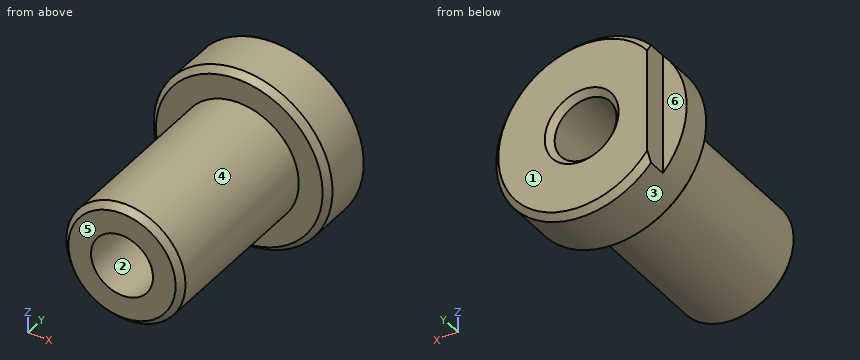
```python
from build123d import *

# Parameters (mm, degrees)
SKETCH1_R           = 5
SKETCH1_R_2         = 2.6
BOSS_EXTRUDE1_DEPTH = 15
SKETCH2_R           = 7.5
SKETCH2_R_2         = 2.6
BOSS_EXTRUDE2_DEPTH = 5
CHAMFER1_SIZE       = 0.5
SKETCH3_W           = 5
SKETCH3_H           = 5
CUT_EXTRUDE1_DEPTH  = 25


with BuildPart() as part:
    # Sketch1 → Boss-Extrude1 (new body)
    with BuildSketch(Plane(origin=(0, 0, 0), x_dir=(1, 0, 0), z_dir=(0, 1, 0))):
        with Locations(Location((0, 0, 0), (0, 0, 270))):
            Circle(SKETCH1_R)
        with Locations(Location((0, 0, 0), (0, 0, 270))):
            Circle(SKETCH1_R_2, mode=Mode.SUBTRACT)
    extrude(amount=BOSS_EXTRUDE1_DEPTH)

    # Sketch2 → Boss-Extrude2 (add)
    with BuildSketch(Plane(origin=(0, 15, 0), x_dir=(1, 0, 0), z_dir=(0, 1, 0))):
        with Locations(Location((0, 0, 0), (0, 0, 270))):
            Circle(SKETCH2_R)
        with Locations(Location((0, 0, 0), (0, 0, 270))):
            Circle(SKETCH2_R_2, mode=Mode.SUBTRACT)
    extrude(amount=BOSS_EXTRUDE2_DEPTH)

    # Chamfer1
    chamfer1_edges = [part.edges().sort_by_distance(p)[0] for p in [
        (0, 20, -7.5),
        (0, 15, -7.5),
        (0, 20, -2.6),
        (0, 0, -5),
    ]]
    chamfer(chamfer1_edges, length=CHAMFER1_SIZE)

    # Sketch3 → Cut-Extrude1 (cut, symmetric)
    with BuildSketch(Plane.XY):
        with Locations((-8, 20.5)):
            Rectangle(SKETCH3_W, SKETCH3_H)
    extrude(amount=CUT_EXTRUDE1_DEPTH, both=True, mode=Mode.SUBTRACT)


solid = part.part
```
CAD build for the part. Positions are in the model's coordinates, mm. Face numbers are marked on the shaded views. A direction names the side the tool comes from. Round coordinates to 2 decimals unless told otherwise and drop trailing zeros. Order: outer loops, then holes, each group sorted by start corner. A loop starts at its lowest first (then second) coordinate and runs counter-clockwise, first axis right, second up.
Item 1: Saw through at B-B on x = 0. Write the cut outline in (y, z), then the cut area to 3 significant figures.
Item 2: Mould opens along X. For the marked faces 1, 2 and 3 say: pulls with the +X half, pulls with the -X half, needs draft (parallel to the pull), parting line crosses it, or undercut.
Item 3: Saw through at A-A on z = 0. Write the cut outline in (x, y), then the cut area to 3 significant figures.
Item 4: Saw through at C-C on y = 7.5. Write the cut outline in (x, z), then the cut area to 3 significant figures.
Item 5: Tool access for the marked faces 4, 5 and 6: list every direction of +Z, -Z, +X, -X, +Y, -Y with a clear straight run to the whole face (end or side of a thin tool).
Item 6: Saw through at D-D on y = 17.75. Write the cut outline in (x, z), then the cut area to 3 significant figures.
Item 7: Probe line 1 along X through (y, z) = (12.75, 0); line 2 along Z through (x, y) = (-6, 17); line 3 along Y through (x, z) = (-5, -3). List the from-to ranges inside material, lowest first.
Item 8: Pin check, flat tips, straight feed: pin 1 (6 mm diameter, centred on y = 8, z = -2, fed in from +X); pin 2 (1 mm diameter, centred on x = 1.5, y = 6, fed in from +Z); pin 3 (4 mm diameter, centred on x = -2.5, y = 5, fed in from +Z); pin 4 (4 mm diameter, centred on x = 0, z = 0, fed in from -Y). Stop position of each tip, or through.
Reported:
1. outline: (0, -4.5) - (0.5, -5) - (15, -5) - (15, -7) - (15.5, -7.5) - (19.5, -7.5) - (20, -7) - (20, -3.1) - (19.5, -2.6) - (0, -2.6) - close; (0, 2.6) - (19.5, 2.6) - (20, 3.1) - (20, 7) - (19.5, 7.5) - (15.5, 7.5) - (15, 7) - (15, 5) - (0.5, 5) - (0, 4.5) - close
1. area: 120 mm2
2. face 1: needs draft
2. face 2: undercut
2. face 3: parting line crosses it
3. outline: (-7.5, 15.5) - (-7, 15) - (-5, 15) - (-5, 0.5) - (-4.5, 0) - (-2.6, 0) - (-2.6, 19.5) - (-3.1, 20) - (-5.5, 20) - (-5.5, 18) - (-7.5, 18) - close; (2.6, 0) - (4.5, 0) - (5, 0.5) - (5, 15) - (7, 15) - (7.5, 15.5) - (7.5, 19.5) - (7, 20) - (3.1, 20) - (2.6, 19.5) - close
3. area: 116 mm2
4. outline: circle Ø10 at (0, 0); hole circle Ø5.2 at (0, 0)
4. area: 57.3 mm2
5. face 4: -Y
5. face 5: +Z, -Z, +X, -X, -Y
5. face 6: +Z, -Z, -X, +Y
6. outline: circle Ø15 at (0, 0); hole circle Ø5.2 at (0, 0)
6. area: 155 mm2
7. line 1: x = -5 to -2.6, 2.6 to 5
7. line 2: z = -4.5 to 4.5
7. line 3: y = 15 to 20
8. pin 1: stops at x = 5
8. pin 2: stops at z = 4.9
8. pin 3: stops at z = 4.97
8. pin 4: passes through
